```python
from build123d import *

# Parameters (mm, degrees)
SKETCH_1_W                = 140
SKETCH_1_H                = 300
EXTRUDE_1_DEPTH           = 10
HOLE_WIZARD_1_D           = 5.5
HOLE_WIZARD_1_DEPTH       = 14.4
HOLE_WIZARD_1_CBORE_D     = 10
HOLE_WIZARD_1_CBORE_DEPTH = 5.7
HOLE_WIZARD_1_TIP         = 1.652366702
HOLE_WIZARD_M5_1_D        = 4.2
HOLE_WIZARD_M5_2_D        = 4.2
HOLE_WIZARD_M5_2_DEPTH    = 12.4
HOLE_WIZARD_M5_2_TIP      = 1.2618073
HOLE_WIZARD_M5_3_D        = 4.2
FILLET_1_R                = 5


with BuildPart() as part:
    # 草图1 → 凸台-拉伸1 (new body)
    with BuildSketch(Plane.XY):
        Rectangle(SKETCH_1_W, SKETCH_1_H)
    extrude(amount=EXTRUDE_1_DEPTH)

    # 打孔尺寸(%根据)内六角圆柱头螺钉的类型1
    with Locations(Plane(origin=(0, 0, 0), x_dir=(-1, 0, 0), z_dir=(0, 0, -1))):
        with Locations((0, 110), (0, 10)):
            CounterBoreHole(HOLE_WIZARD_1_D / 2, HOLE_WIZARD_1_CBORE_D / 2, HOLE_WIZARD_1_CBORE_DEPTH, depth=HOLE_WIZARD_1_DEPTH)
            with Locations((0, 0, -(HOLE_WIZARD_1_DEPTH + HOLE_WIZARD_1_TIP / 2))):  # 118° drill point
                Cone(0, HOLE_WIZARD_1_D / 2, HOLE_WIZARD_1_TIP, mode=Mode.SUBTRACT)

    # M5 螺纹孔1 (through all)
    with Locations(Plane(origin=(0, 0, 0), x_dir=(-1, 0, 0), z_dir=(0, 0, -1))):
        with Locations((-4.800000353, -65.5), (63.199999647, -65.5), (-4.800000353, 34.5), (63.199999647, 34.5), (-4.800000353, 134.5), (63.199999647, 134.5)):
            Hole(HOLE_WIZARD_M5_1_D / 2)

    # M5 螺纹孔2
    with Locations(Plane(origin=(0, -150, 0), x_dir=(-1, 0, 0), z_dir=(0, -1, 0))):
        with Locations((-50, -5), (50, -5)):
            Hole(HOLE_WIZARD_M5_2_D / 2, depth=HOLE_WIZARD_M5_2_DEPTH)
            with Locations((0, 0, -(HOLE_WIZARD_M5_2_DEPTH + HOLE_WIZARD_M5_2_TIP / 2))):  # 118° drill point
                Cone(0, HOLE_WIZARD_M5_2_D / 2, HOLE_WIZARD_M5_2_TIP, mode=Mode.SUBTRACT)

    # M5 螺纹孔3 (through all)
    with Locations(Plane.XY.offset(10)):
        with Locations((45, 90), (45, 30), (45, -70)):
            Hole(HOLE_WIZARD_M5_3_D / 2)

    # 圆角1
    fillet_1_edges = [part.edges().sort_by_distance(p)[0] for p in [
        (-70, 150, 5),
        (70, 150, 5),
    ]]
    fillet(fillet_1_edges, radius=FILLET_1_R)


solid = part.part
```
Geometry check sheet. Reference: the model listing, model coordinates, mm. A direction names the side the tool comes from. Give positions to 0.01 mm unless a question says otherwise; leave off trailing zeros. Write each loop counter-clockwise with the first axis right and the second up, starting at its lowest first coordinate (ties: lowest second). Pieces come first, ordered by that corner, then holes.
1) Gauge pin test, flat end, axial feed: pin 1 (8 mm diameter, centred on x = 0, y = 110, fed in from -Z). Record the tip position at first contact, or that the pin passes through.
2) Section check B-B, the plane x = 0. Record the boundary of the cut face in (y, z), and give its area (3 significant figures).
3) Section check A-A, the plane y = 110. Record the boundary of the cut face in (x, z), and give its area (3 significant figures).
4) Release check for a two-part mould opening along Y. For faces 3 (the flat face through (-1, 2, 0)), 4 (the cylindrical face through (-0.596, 107.315, 7.88)), 5 (the flat face through (-1, -150, 5)) record: pulls with the +Y half, pulls with the -Y half, needs draft (parallel to the pull), parting line crosses it, or undercut.
5) Material ranges on L1, parallel to Y at x = 45, z = 3.75; L2, parallel to Y at x = 0, z = 6.8; L3, parallel to Y at x = 4.8, z = 6.5, recorded low to high.
6) Access from +Z, -Z, +X, -X, +Y, -Y to the whole of each face (thin tool, end or side, straight path). Record for faces 1 (the flat face through (-2.2, 107.8, 5.7)), 2 (the flat face through (-70, -5, 5)).
Computed:
1. pin 1: stops at z = 5.7
2. outline: (-150, 0) - (5, 0) - (5, 5.7) - (7.25, 5.7) - (7.25, 10) - (-150, 10) - close; (12.75, 5.7) - (15, 5.7) - (15, 0) - (105, 0) - (105, 5.7) - (107.25, 5.7) - (107.25, 10) - (12.75, 10) - close; (112.75, 5.7) - (115, 5.7) - (115, 0) - (150, 0) - (150, 10) - (112.75, 10) - close
2. area: 2,840 mm2
3. outline: (-70, 0) - (-5, 0) - (-5, 5.7) - (-2.75, 5.7) - (-2.75, 10) - (-70, 10) - close; (2.75, 5.7) - (5, 5.7) - (5, 0) - (70, 0) - (70, 10) - (2.75, 10) - close
3. area: 1,320 mm2
4. face 3: needs draft
4. face 4: undercut
4. face 5: pulls with the -Y half
5. L1: y = -150 to -72.1, -67.9 to 27.9, 32.1 to 87.9, 92.1 to 150
5. L2: y = -150 to 7.25, 12.75 to 107.25, 112.75 to 150
5. L3: y = -150 to -67.6, -63.4 to 32.4, 36.6 to 132.4, 136.6 to 150
6. face 1: -Z
6. face 2: +Z, -Z, -X, +Y, -Y
